Answer from the drawing. Dimensions are ordinates in mm from the lowest x, y and z of the part. A direction names the side the tool comes from. Coordinates: 2 decimals unless noted, no trailing zeros. Order: outer loops, then holes, each group sorted by start corner. A loop starts at its lowest first (then second) coordinate and runs counter-clockwise, first axis right, second up. Notation, with made-up numbers: (39, 12) - (58, 12) arc R27 cw to (58, 35) - close; hole circle Ø10 at (-1, 81). An arc over 180 degrees is marked (long way). Answer as a JSON object with one key per item and string values. Group by question number.
1) Section A-A (z = 65) is taken. Give the vertices of the cut face in (x, y), plus the area to 3 significant figures.
2) Section D-D (y = 79) is taken. Give the vertices of the cut face in (x, z).
3) Section B-B (x = 70) is taken. Give the vertices of the cut face in (y, z), plus the area to 3 significant figures.
4) The mould has two halves that part along X. Classify the marked faces 1, 2, 3 and 4: released by +X, released by -X, zero draft, split by the parting line, or undercut.
5) Each of these flat-tipped pins is pushed along its axis until it touches: P1, Ø6, axis at x = 124, y = 28, coming from the +Z side; P2, Ø11.5, axis at y = 10, z = 10, coming from the +X side; P3, Ø10, axis at x = 8.5, z = 59.5, coming from the +Y side; P4, Ø4, axis at y = 74.5, z = 61, coming from the -X side. Where does it stop, or does it pass through?
6) A tool of negligible diameter and unlimited length cuts with its end or side. For the marked faces 5, 6, 7, 8 and 9, from which of +Z, -Z, +X, -X, +Y, -Y can it reach the whole face along a straight path? Write none if from no direction.
7) Section C-C (y = 28) is taken. Give the vertices of the cut face in (x, z), plus the area to 3 significant figures.
8) Find the intervals of material crossed by line 1 along Y through (x, z) = (124, 65); line 2 along Z through (x, y) = (31.5, 24); line 3 along Y through (x, z) = (70, 73.5), in increasing order.
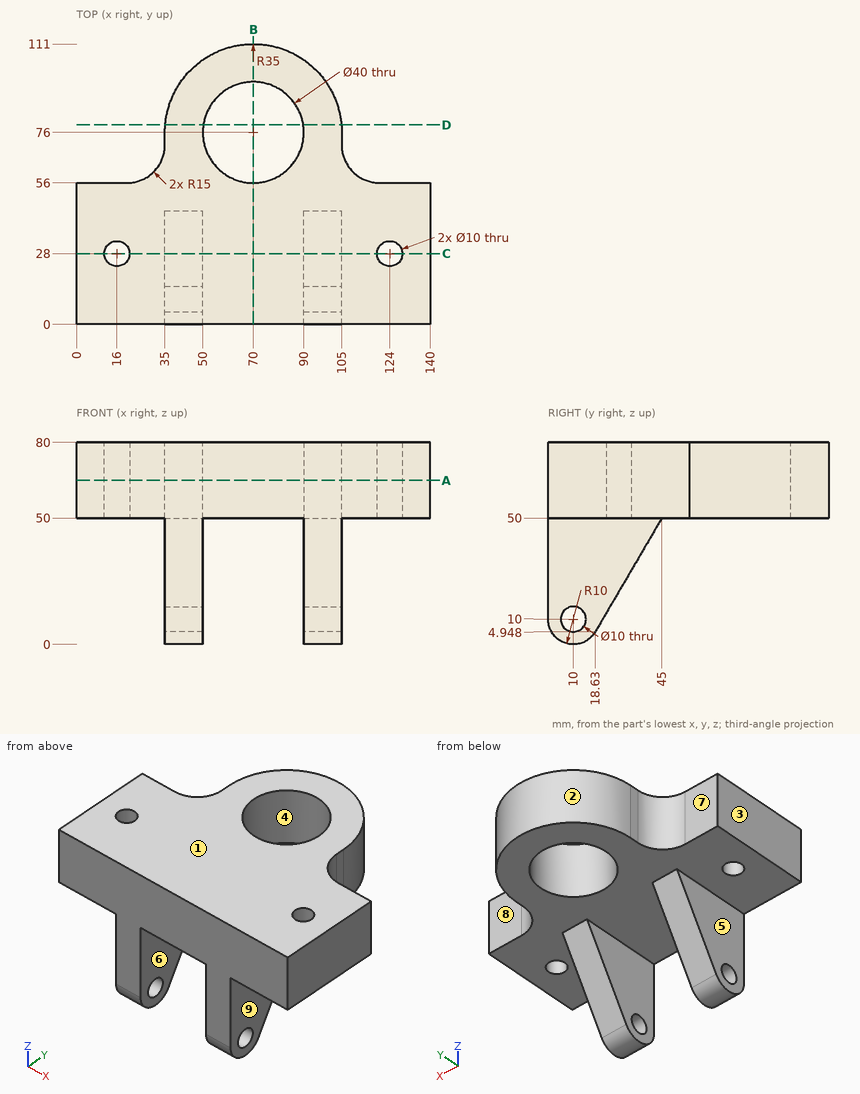
Report:
{
 "1": {"outline": "(0, 0) - (140, 0) - (140, 56) - (120, 56) arc R15 cw to (105, 71) - (105, 76) arc R35 ccw to (35, 76) - (35, 71) arc R15 cw to (20, 56) - (0, 56) - close; hole circle Ø10 at (16, 28); hole circle Ø40 at (70, 76); hole circle Ø10 at (124, 28)", "area": "9,850 mm²"},
 "2": {"outline": "(35.13, 50) - (50.23, 50) - (50.23, 80) - (35.13, 80) - close; (89.77, 50) - (104.87, 50) - (104.87, 80) - (89.77, 80) - close"},
 "3": {"outline": "(0, 50) - (56, 50) - (56, 80) - (0, 80) - close; (96, 50) - (111, 50) - (111, 80) - (96, 80) - close", "area": "2,130 mm²"},
 "4": {"face 1": "zero draft", "face 2": "split by the parting line", "face 3": "released by -X", "face 4": "undercut"},
 "5": {"P1": "passes through", "P2": "stops at x = 105", "P3": "stops at y = 56", "P4": "stops at x = 35"},
 "6": {"face 5": "-Z, -X, +Y, -Y", "face 6": "-Z, +Y, -Y", "face 7": "+Z, -Z, -X, +Y", "face 8": "+Z, -Z, +X, +Y", "face 9": "-Z, +X, +Y, -Y"},
 "7": {"outline": "(0, 50) - (11, 50) - (11, 80) - (0, 80) - close; (21, 50) - (35, 50) - (35, 20.96) - (50, 20.96) - (50, 50) - (90, 50) - (90, 20.96) - (105, 20.96) - (105, 50) - (119, 50) - (119, 80) - (21, 80) - close; (129, 50) - (140, 50) - (140, 80) - (129, 80) - close", "area": "4,470 mm²"},
 "8": {"line 1": "y = 0 to 23, 33 to 56", "line 2": "z = 50 to 80", "line 3": "y = 0 to 56, 96 to 111"}
}
